from build123d import *

# Parameters (mm, degrees)
SKETCH1_W           = 400
SKETCH1_H           = 1000
BOSS_EXTRUDE1_DEPTH = 10
SKETCH2_R           = 10
CUT_EXTRUDE1_DEPTH  = 42
CUT_EXTRUDE2_DEPTH  = 20


with BuildPart() as part:
    # Sketch1 → Boss-Extrude1 (new body)
    with BuildSketch(Plane.XY):
        Rectangle(SKETCH1_W, SKETCH1_H)
    extrude(amount=BOSS_EXTRUDE1_DEPTH)

    # Sketch2 → Cut-Extrude1 (cut)
    with BuildSketch(Plane(origin=(0, 0, 0), x_dir=(-1, 0, 0), z_dir=(0, 0, -1))):
        with Locations((-180, 480)):
            Circle(SKETCH2_R)
        with Locations((180, 480)):
            Circle(SKETCH2_R)
        with Locations((180, -480)):
            Circle(SKETCH2_R)
        with Locations((-180, -480)):
            Circle(SKETCH2_R)
    extrude(amount=-CUT_EXTRUDE1_DEPTH, mode=Mode.SUBTRACT)

    # Sketch3 → Cut-Extrude2 (cut)
    with BuildSketch(Plane.XY.offset(10)):
        with BuildLine():
            Line((100, 200), (100, -200))
            ThreePointArc((100, -200), (0, -300), (-100, -200))
            Line((-100, -200), (-100, 200))
            ThreePointArc((-100, 200), (0, 300), (100, 200))
        make_face()
    extrude(amount=-CUT_EXTRUDE2_DEPTH, mode=Mode.SUBTRACT)


solid = part.part
Could you check a few things on this model? Use its own coordinates, in mm. A direction names the side the tool comes from. Give positions to 0.01 mm unless a question says otherwise; leave off trailing zeros. Write each loop counter-clockwise with the first axis right and the second up, starting at its lowest first coordinate (ties: lowest second). Pieces come first, ordered by that corner, then holes. Notation, with made-up numbers: (-12.5, 34) -> (21.5, 34) arc R16 cw to (21.5, 57) -> close; hole circle Ø10 at (-29.75, 7). An arc over 180 degrees is marked (long way). Answer as CSV lines item,"result". Start each with the question number.
(1) If we mould it in two halves opening along Y, with no side actions, what happens to faces 3 (the face through (-136, 7, 10)), 4 (the face through (181.302, -470.085, 4.93))? For each: +Y half, -Y half, draft (parallel to the pull), parting line (faces both ways), or undercut.
(2) Which directions (+Z, -Z, +X, -X, +Y, -Y) give clear straight access to the entire face, cutting with the end or side of a thin tool? Please do faces 1 (the face through (2.199, -299.976, 5.07)), 2 (the face through (-136, 7, 0)).
(3) If we section it at C-C, the plane x = 180: Write out the boundary of the cut face in (y, z).
(4) If we section it at A-A, the plane x = 0: Write out the boundary of the cut face in (y, z), and give its area (3 significant figures).
(5) If we section it at B-B, the plane y = 67: Write out the boundary of the cut face in (x, z).
(6) Please list where these lines run through material, in increasing order: line 1 (Y direction, x = 178, z = 4); line 2 (Y direction, x = -180, z = 5.75); line 3 (X direction, y = -59, z = 0.5).
(7) If we section it at D-D, the plane z = 5: Write out the boundary of the cut face in (x, y), and give its area (3 significant figures).
Answer list:
1,face 3,"draft"
1,face 4,"undercut"
2,face 1,"+Z, -Z"
2,face 2,"-Z, +X, -X, +Y, -Y"
3,outline,"(-500, 0) -> (-490, 0) -> (-490, 10) -> (-500, 10) -> close; (-470, 0) -> (470, 0) -> (470, 10) -> (-470, 10) -> close; (490, 0) -> (500, 0) -> (500, 10) -> (490, 10) -> close"
4,outline,"(-500, 0) -> (-300, 0) -> (-300, 10) -> (-500, 10) -> close; (300, 0) -> (500, 0) -> (500, 10) -> (300, 10) -> close"
4,area,"4,000 mm^2"
5,outline,"(-200, 0) -> (-100, 0) -> (-100, 10) -> (-200, 10) -> close; (100, 0) -> (200, 0) -> (200, 10) -> (100, 10) -> close"
6,line 1,"-500 to -489.8, -470.2 to 470.2, 489.8 to 500"
6,line 2,"-500 to -490, -470 to 470, 490 to 500"
6,line 3,"-200 to -100, 100 to 200"
7,outline,"(-200, -500) -> (200, -500) -> (200, 500) -> (-200, 500) -> close; hole circle Ø20 at (-180, -480); hole circle Ø20 at (-180, 480); hole (-100, -200) arc R100 ccw to (100, -200) -> (100, 200) arc R100 ccw to (-100, 200) -> close; hole circle Ø20 at (180, -480); hole circle Ø20 at (180, 480)"
7,area,"287,000 mm^2"
